from build123d import *

# Parameters (mm, degrees)
SKETCH_1_R      = 35
EXTRUDE_1_DEPTH = 40
SKETCH_2_R      = 5
EXTRUDE_2_DEPTH = 33
EXTRUDE_START   = 33
SKETCH_3_R      = 5
EXTRUDE_3_DEPTH = 33


with BuildPart() as part:
    # 草图1 → 凸台-拉伸1 (new body)
    with BuildSketch(Plane.XY):
        Circle(SKETCH_1_R)
    extrude(amount=EXTRUDE_1_DEPTH)

    # 草图2 → 凸台-拉伸2 (add)
    with BuildSketch(Plane.XY.offset(40)):
        Circle(SKETCH_2_R)
    extrude(amount=EXTRUDE_2_DEPTH)

    # 草图3 → 凸台-拉伸3 (add)
    with BuildSketch(Plane(origin=(0, 0, 0), x_dir=(-1, 0, 0), z_dir=(0, 0, -1)).offset(EXTRUDE_START)):
        with Locations(Location((0, 0, 0), (0, 0, 180))):
            Circle(SKETCH_3_R)
    extrude(amount=-EXTRUDE_3_DEPTH)


solid = part.part
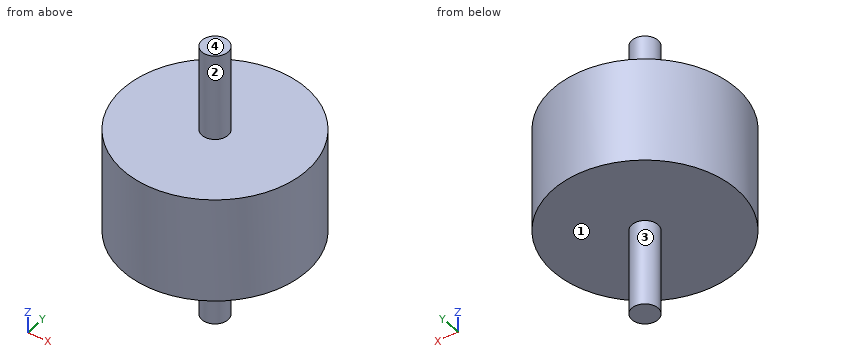
The model under review builds one solid part; all positions refer to its coordinate system, in mm. Face numbers are marked on the shaded views. A direction names the side the tool comes from. Round coordinates to 2 decimals unless told otherwise and drop trailing zeros. Order: outer loops, then holes, each group sorted by start corner. A loop starts at its lowest first (then second) coordinate and runs counter-clockwise, first axis right, second up. Notation, with made-up numbers: (41, 51) -> (65, 51) arc R25 ccw to (65, 71) -> close; hole circle Ø7 at (36, 2.5). An arc over 180 degrees is marked (long way). Return JSON: item names as keys, results as strings.
1. For L1, parallel to Z at x = 23, y = -7; L2, parallel to Y at x = 2, z = 48; L3, parallel to Y at x = 11.5, z = 14, list the stretches that pass through material, from the lowest coordinate up. Write a range as [from, to].
Answer block:
{"L1": "z = [0, 40]", "L2": "y = [-4.58, 4.58]", "L3": "y = [-33.06, 33.06]"}
2. The part is to be moulded in two halves that separate along Y. For the marked faces 1 and 2, say which applies: +Y half, -Y half, draft (parallel to the pull), parting line (faces both ways), or undercut.
Answer block:
{"face 1": "draft", "face 2": "parting line"}
3. Take a section at C-C (z = -19). Write out the cut boundary in (x, y), then the cut area to 3 significant figures.
Answer block:
{"outline": "circle Ø10 at (0, 0)", "area": "78.5 mm²"}
4. Insertion check: P1, Ø12, axis at x = -7.5, z = 0, coming from the -Y side; P2, Ø5, axis at y = -3.5, z = 60, coming from the -X side; P3, Ø4, axis at x = -18, z = -0.5, coming from the +Y side. Each pin has a flat end and moves straight along its axis. Give the tip position at first contact, or say it passes through.
Answer block:
{"P1": "stops at y = -34.97", "P2": "stops at x = -4.9", "P3": "stops at y = 31.1"}
5. Take a section at A-A (x = 0). Write out the cut boundary in (y, z).
Answer block:
{"outline": "(-35, 0) -> (-5, 0) -> (-5, -33) -> (5, -33) -> (5, 0) -> (35, 0) -> (35, 40) -> (5, 40) -> (5, 73) -> (-5, 73) -> (-5, 40) -> (-35, 40) -> close"}
6. For the marked faces 3 and 4, list the 3-axis set-ups (+Z, -Z, +X, -X, +Y, -Y) from which the entire face can be reached by the end or side of a thin tool; tool diameter is ignored.
Answer block:
{"face 3": "-Z", "face 4": "+Z, +X, -X, +Y, -Y"}
7. Take a section at D-D (y = 31). Write out the cut boundary in (x, z).
Answer block:
{"outline": "(-16.25, 0) -> (16.25, 0) -> (16.25, 40) -> (-16.25, 40) -> close"}
